Could you check a few things on this model? Use its own coordinates, in mm. A direction names the side the tool comes from. Round coordinates to 2 decimals unless told otherwise and drop trailing zeros. Order: outer loops, then holes, each group sorted by start corner. A loop starts at its lowest first (then second) coordinate and runs counter-clockwise, first axis right, second up.
```python
from build123d import *

# Parameters (mm, degrees)
CLAMP_LOOP_30MM_DEPTH   = 15
SUPPORT_WEB_18MM_DEPTH  = 9
MOUNTING_LUG_DEPTH      = 2
MOUNTING_LUG_DEPTH_BACK = 9
SKETCH1_4_R             = 11


with BuildPart() as part:
    # Bracket Profile Sketch → Clamp Loop 30mm (new, symmetric)
    with BuildSketch(Plane.XY):
        with BuildLine():
            ThreePointArc((-161.958144077, 21.543307087), (-152.82526794, -33.65504728), (-124.10035648, -81.666995927))
            ThreePointArc((-124.10035648, -81.666995927), (-91.629362444, -83.573444545), (-89.722913826, -51.102450509))
            ThreePointArc((-89.722913826, -51.102450509), (-109.638852439, -17.814166114), (-115.970979893, 20.456692913))
            ThreePointArc((-115.970979893, 20.456692913), (-138.421254898, 43.993582092), (-161.958144077, 21.543307087))
        make_face()
        with BuildLine():
            ThreePointArc((-122.969026617, 20.622047244), (-138.586609229, 36.995535368), (-154.960097353, 21.377952756))
            ThreePointArc((-154.960097353, 21.377952756), (-146.253422103, -31.244478407), (-118.869006511, -77.01586945))
            ThreePointArc((-118.869006511, -77.01586945), (-96.280488921, -78.342094576), (-94.954263795, -55.753576986))
            ThreePointArc((-94.954263795, -55.753576986), (-116.210698276, -20.224734987), (-122.969026617, 20.622047244))
        make_face(mode=Mode.SUBTRACT)
    extrude(amount=CLAMP_LOOP_30MM_DEPTH, both=True)

    # Sketch1_3 → Support Web 18mm (add, symmetric)
    with BuildSketch(Plane.XY):
        with BuildLine():
            Line((-23, -44), (-23, 44))
            Line((-23, 44), (-138.964561985, 44))
            ThreePointArc((-138.964561985, 44), (-122.51013913, 37.070219927), (-115.970979893, 20.456692913))
            ThreePointArc((-115.970979893, 20.456692913), (-115.999941726, 18.110094916), (-115.975948196, 15.76344086))
            ThreePointArc((-115.975948196, 15.76344086), (-112.839858129, 23.694083749), (-104.978492137, 27))
            Line((-104.978492137, 27), (-65.39696962, 27))
            ThreePointArc((-65.39696962, 27), (-42.299981307, 11.567085809), (-47.71930009, -15.67766953))
            Line((-47.71930009, -15.67766953), (-78.190423053, -46.148792492))
            ThreePointArc((-78.190423053, -46.148792492), (-86.706172416, -49.345862018), (-94.717571561, -45.038110339))
            ThreePointArc((-94.717571561, -45.038110339), (-92.277527324, -48.11746068), (-89.722913826, -51.102450509))
            ThreePointArc((-89.722913826, -51.102450509), (-83.921522259, -67.059044464), (-90.648179186, -82.648179186))
            Line((-90.648179186, -82.648179186), (-52, -44))
            Line((-52, -44), (-23, -44))
        make_face()
    extrude(amount=SUPPORT_WEB_18MM_DEPTH, both=True)

    # Sketch1_4 → Mounting Lug (add, two sides: drawn at the far end of the back side and taken through both)
    with BuildSketch(Plane.XY.offset(-MOUNTING_LUG_DEPTH_BACK)):
        with BuildLine():
            ThreePointArc((35, 26.664583252), (19.528931575, 39.428680317), (0, 44))
            Line((0, 44), (-23, 44))
            Line((-23, 44), (-23, -44))
            Line((-23, -44), (0, -44))
            ThreePointArc((0, -44), (19.528931575, -39.428680317), (35, -26.664583252))
            Line((35, -26.664583252), (35, 26.664583252))
        make_face()
        Circle(SKETCH1_4_R, mode=Mode.SUBTRACT)
    extrude(amount=MOUNTING_LUG_DEPTH + MOUNTING_LUG_DEPTH_BACK)


solid = part.part
```
Q1. I need wall thicknesses on L1, parallel to X at y = -30.5, z = 2.5; L2, parallel to X at y = -28, z = -4; L3, parallel to Y at x = -98.5, z = 4. Which ranges of each line are inside material? Lowest first, please.
Q2. For P1, Ø1, axis at y = 13.5, z = -11, coming from the +X side; P2, Ø2, axis at y = -71.5, z = -11.5, coming from the -X side; P3, Ø6, axis at x = 4, z = -5.5, coming from the +Y side; P4, Ø17.5, axis at x = 0, y = 0, coming from the +Z side, each with a flat end and sliding along its axis, tell me the tip position at first contact or that it passes through.
Q3. Imagine slicing it at A-A, the plane y = 0. Please give me the cut outline in (x, z), then the cut area to 3 significant figures.
Q4. Imagine slicing it at D-D, the plane y = -30.5. Please give me the cut outline in (x, z), then the cut area to 3 significant figures.
Q5. For faces 1 (the flat face through (-26, -44, -2)), 2 (the flat face through (12, 1, 2)), 3 (the cylindrical face through (-98.902, -87.945, 0.21)), 4 (the cylindrical face through (-146.51, -30.54, 0.21)), 5 (the flat face through (-114, -22, -15)), which set-ups out of +Z, -Z, +X, -X, +Y, -Y let a thin tool reach every point of the face, with its end or its side?
Q6. Imagine slicing it at C-C, the plane z = 5.5. Please give me the cut outline in (x, y).
Q7. Imagine slicing it at B-B, the plane x = -45. Please give me the cut outline in (y, z).
Filled in:
1. L1: x = -153.94 to -146.52, -111.84 to -104, -62.54 to -23
1. L2: x = -154.77 to -147.4, -113.02 to -105.27, -60.04 to 33.94
1. L3: y = -87.79 to -80, -51.56 to -39.74, 27 to 44
2. P1: stops at x = -115.88
2. P2: stops at x = -133.11
2. P3: stops at y = 43.99
2. P4: passes through
3. outline: (-160.92, -15) - (-153.86, -15) - (-153.86, 15) - (-160.92, 15) - close; (-121.53, -15) - (-114.43, -15) - (-114.43, 15) - (-121.53, 15) - close; (-40.48, -9) - (-11, -9) - (-11, 2) - (-23, 2) - (-23, 9) - (-40.48, 9) - close; (11, -9) - (35, -9) - (35, 2) - (11, 2) - close
3. area: 1,140 mm2
4. outline: (-153.94, -15) - (-146.52, -15) - (-146.52, 15) - (-153.94, 15) - close; (-111.84, -15) - (-104, -15) - (-104, 15) - (-111.84, 15) - close; (-62.54, -9) - (31.71, -9) - (31.71, 2) - (-23, 2) - (-23, 9) - (-62.54, 9) - close
4. area: 1,770 mm2
5. face 1: +Z, -Z, +X, -Y
5. face 2: +Z, +X, +Y, -Y
5. face 3: none
5. face 4: +Z, -Z
5. face 5: -Z, +X, -X, +Y, -Y
6. outline: (-161.96, 21.54) arc R150 ccw to (-124.1, -81.67) arc R23 ccw to (-90.65, -82.65) - (-52, -44) - (-23, -44) - (-23, 44) - (-138.96, 44) arc R23 ccw to start; hole (-154.96, 21.38) arc R143 ccw to (-118.87, -77.02) arc R16 ccw to (-94.95, -55.75) arc R111 cw to (-122.97, 20.62) arc R16 ccw to start; hole (-115.98, 15.76) arc R104 ccw to (-94.72, -45.04) arc R11 ccw to (-78.19, -46.15) - (-47.72, -15.68) arc R25 ccw to (-65.4, 27) - (-104.98, 27) arc R11 ccw to start
7. outline: (-44, -9) - (-12.46, -9) - (-12.46, 9) - (-44, 9) - close; (16.46, -9) - (44, -9) - (44, 9) - (16.46, 9) - close
